```python
from build123d import *

# Parameters (mm, degrees)
SKETCH_1_R          = 7.5
EXTRUDE_1_DEPTH     = 545
FILLET_1_R          = 2
SKETCH_2_W          = 5
SKETCH_2_H          = 6.769617338
CUT_EXTRUDE_2_DEPTH = 20
SKETCH_3_R          = 2.5
CUT_EXTRUDE_3_DEPTH = 546.194919376


with BuildPart() as part:
    # 草图1 → 拉伸1 (new, symmetric)
    with BuildSketch(Plane.XY):
        Circle(SKETCH_1_R)
    extrude(amount=EXTRUDE_1_DEPTH, both=True)

    # 圆角1
    fillet_1_edges = [part.edges().sort_by_distance(p)[0] for p in [
        (-7.5, 0, -545),
        (-7.5, 0, 545),
    ]]
    fillet(fillet_1_edges, radius=FILLET_1_R)

    # 草图2 → 拉伸2 (cut)
    with BuildSketch(Plane(origin=(0, 0, -545), x_dir=(-1, 0, 0), z_dir=(0, 0, -1))):
        with Locations((0, 8.384808669)):
            Rectangle(SKETCH_2_W, SKETCH_2_H)
    extrude(amount=-CUT_EXTRUDE_2_DEPTH, mode=Mode.SUBTRACT)

    # 草图3 → 拉伸3 (cut, through all)
    with BuildSketch(Plane(origin=(0, 5, 0), x_dir=(1, 0, 0), z_dir=(0, 1, 0))):
        with Locations((0, 525)):
            Circle(SKETCH_3_R)
    extrude(amount=CUT_EXTRUDE_3_DEPTH, mode=Mode.SUBTRACT)


solid = part.part
```
For this review, take the finished solid that the model builds, in its own axes (mm). Round coordinates to 2 decimals unless told otherwise and drop trailing zeros. Write each loop counter-clockwise with the first axis right and the second up, starting at its lowest first coordinate (ties: lowest second). Pieces come first, ordered by that corner, then holes. Notation, with made-up numbers: (30.5, 66) -> (59.5, 66) arc R19 cw to (59.5, 70) -> close; hole circle Ø8 at (39.25, 83). An arc over 180 degrees is marked (long way). Use one line per item in the form item = value.
Q1. Clearance check with flat-ended pins moving along their axes: pin 1 Ø0.6 at (y, z) = (6.5, -538.5) entering from -X; pin 2 Ø5.5 at (x, z) = (-0.5, -539) entering from +Y; pin 3 Ø0.6 at (y, z) = (6, -535.5) entering from +X. State where each tip first meets the part, or that it passes through.
Resolved:
pin_1 = -4.22
pin_2 = 7.07
pin_3 = 4.87
Q2. Consider section A-A (z = -447.5). State the section outline as (x, y) points, then the cut area to 3 significant figures.
Resolved:
outline = circle Ø15 at (0, 0)
area = 177 mm²
Q3. To check wall thickness, follow probe 1 along Y at (x, z) = (1, 101.5); probe 2 along X at (y, z) = (-0.25, -184). State the ranges of each line that lie inside material, in increasing order. Write a range as from..to.
Resolved:
probe_1 = -7.43..7.43
probe_2 = -7.5..7.5
